Check sheet for the modelled part. Datum: model origin and axes. Units: mm. A direction names the side the tool comes from. Coordinates: 2 decimals unless noted, no trailing zeros. Order: outer loops, then holes, each group sorted by start corner. A loop starts at its lowest first (then second) coordinate and runs counter-clockwise, first axis right, second up. Notation, with made-up numbers: (38, -12) -> (57, -12) arc R16 ccw to (57, -8) -> close; hole circle Ø3 at (25, 7.25). An arc over 180 degrees is marked (long way). Put each result on its own line as item: value. Start each with the question number.
```python
from build123d import *

# Parameters (mm, degrees)
SKETCH_1_R             = 26
EXTRUDE_1_DEPTH        = 70
SKETCH_2_R             = 11
EXTRUDE_2_DEPTH        = 2
SKETCH_3_R             = 4
EXTRUDE_3_DEPTH        = 24
HOLE_WIZARD_M2_1_D     = 1.6
HOLE_WIZARD_M2_1_DEPTH = 5.2
HOLE_WIZARD_M2_1_TIP   = 0.480688495


with BuildPart() as part:
    # 草图1 → 凸台-拉伸1 (new body)
    with BuildSketch(Plane.XY):
        Circle(SKETCH_1_R)
    extrude(amount=EXTRUDE_1_DEPTH)

    # 草图2 → 凸台-拉伸2 (add)
    with BuildSketch(Plane.XY.offset(70)):
        Circle(SKETCH_2_R)
    extrude(amount=EXTRUDE_2_DEPTH)

    # 草图3 → 凸台-拉伸3 (add)
    with BuildSketch(Plane.XY.offset(72)):
        Circle(SKETCH_3_R)
    extrude(amount=EXTRUDE_3_DEPTH)

    # M2 螺纹孔1
    with Locations(Plane.XY.offset(70)):
        with Locations((0, 21.5), (15.202795796, 15.202795796), (21.5, 0), (15.202795796, -15.202795796), (0, -21.5), (-15.202795796, -15.202795796), (-21.5, 0), (-15.202795796, 15.202795796)):
            Hole(HOLE_WIZARD_M2_1_D / 2, depth=HOLE_WIZARD_M2_1_DEPTH)
            with Locations((0, 0, -(HOLE_WIZARD_M2_1_DEPTH + HOLE_WIZARD_M2_1_TIP / 2))):  # 118° drill point
                Cone(0, HOLE_WIZARD_M2_1_D / 2, HOLE_WIZARD_M2_1_TIP, mode=Mode.SUBTRACT)


solid = part.part
```
1) Sectioned sample at D-D (y = -5). Record the boundary of the cut face in (x, z).
2) Sectioned sample at B-B (z = 36). Record the boundary of the cut face in (x, y).
3) Gauge pin test, flat ends, axial feed: pin 1 (5 mm diameter, centred on x = 17.5, z = 45.5, fed in from +Y); pin 2 (2 mm diameter, centred on x = 21.5, y = 0, fed in from +Z); pin 3 (1.3 mm diameter, centred on x = 15.2, y = -15.2, fed in from +Z). Record the tip position at first contact, or that the pin passes through.
4) Access from +Z, -Z, +X, -X, +Y, -Y to the whole of each face (thin tool, end or side, straight path). Record for faces 1 (the cylindrical face through (-0.867, -3.905, 83.832)), 2 (the flat face through (0, 0, 96)).
5) Scan lines: line 1 along Y through (x, z) = (0, 68); line 2 along Z through (x, y) = (18, -15); line 3 along Y through (x, z) = (-21.5, 66.65). Record each from-to range of solid material in increasing order. Write a range as [from, to].
6) Sectioned sample at C-C (x = -12). Record the boundary of the cut face in (y, z).
7) Sectioned sample at A-A (y = 7). Record the boundary of the cut face in (x, z).
Entries:
1. outline: (-25.51, 0) -> (25.51, 0) -> (25.51, 70) -> (9.8, 70) -> (9.8, 72) -> (-9.8, 72) -> (-9.8, 70) -> (-25.51, 70) -> close
2. outline: circle Ø52 at (0, 0)
3. pin 1: stops at y = 21.24
3. pin 2: stops at z = 70
3. pin 3: stops at z = 64.71
4. face 1: +Z
4. face 2: +Z, +X, -X, +Y, -Y
5. line 1: y = [-26, -22.3], [-20.7, 20.7], [22.3, 26]
5. line 2: z = [0, 70]
5. line 3: y = [-14.62, -0.8], [0.8, 14.62]
6. outline: (-23.07, 0) -> (23.07, 0) -> (23.07, 70) -> (-23.07, 70) -> close
7. outline: (-25.04, 0) -> (25.04, 0) -> (25.04, 70) -> (8.49, 70) -> (8.49, 72) -> (-8.49, 72) -> (-8.49, 70) -> (-25.04, 70) -> close
